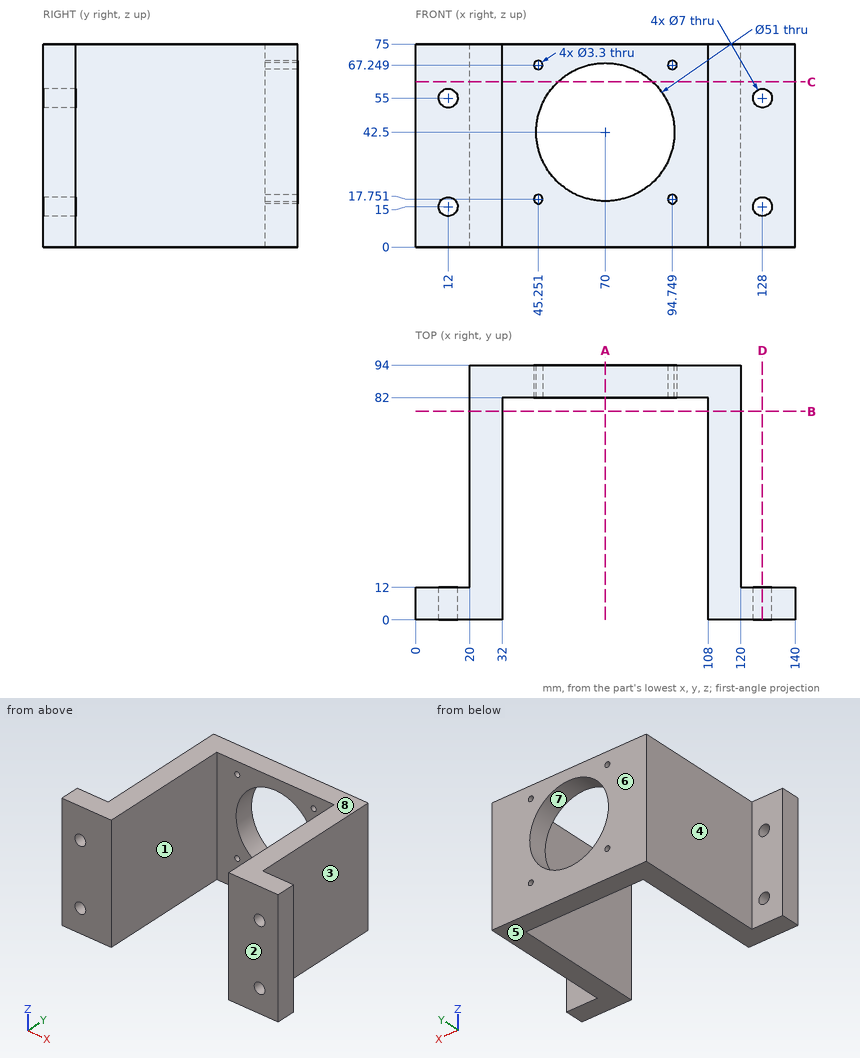
The figure shows three views and two pictorial views of one solid part (mm, origin at its lowest corner). Answer the questions. A direction names the side the tool comes from. Round coordinates to 2 decimals unless told otherwise and drop trailing zeros. Order: outer loops, then holes, each group sorted by start corner. A loop starts at its lowest first (then second) coordinate and runs counter-clockwise, first axis right, second up. Notation, with made-up numbers: M 23.5,43 L 55.5,43 A20 ccw 55.5,61 Z; hole C 25.5,17 d3. An arc over 180 degrees is marked long. Answer in a Markdown table with one row per item. Add a question column.
1) The part is cut by section B-B on y = 77. Determine the outline of the cut face in (x, z), plus the area to 3 significant figures.
2) The part is cut by section D-D on x = 128. Determine the outline of the cut face in (y, z).
3) Which of the six approach directions +Z, -Z, +X, -X, +Y, -Y give full straight-line access (tool end or side, diameter ignored) to the marked faces 1, 2, 3, 4 and 5?
4) The part is cut by section C-C on z = 61. Determine the outline of the cut face in (x, y), plus the area to 3 significant figures.
5) Flat-ended cylindrical pins translate along their axes: pin 1 Ø9 at (x, z) = (128, 55) entering from +Y; pin 2 Ø3 at (y, z) = (25, 25) entering from +X. Find the tip coordinate at first contact, or state that the pin passes through.
6) Determine the mould class of the marked faces 6, 7 and 8 for opening direction Z: pulls with the +Z half, pulls with the -Z half, needs draft (parallel to the pull), parting line crosses it, or undercut.
7) Consider line 1 along X through (y, z) = (5, 15); line 2 along X through (y, z) = (50.5, 69); line 3 along Y through (x, z) = (40, 53.5). Determine where each line is inside the solid, lowest interval first. Write a range as from..to.
8) The part is cut by section A-A on x = 70. Determine the outline of the cut face in (y, z).
Findings below:
| question | item | result |
|---|---|---|
| 1 | outline | M 20,0 L 32,0 L 32,75 L 20,75 Z; M 108,0 L 120,0 L 120,75 L 108,75 Z |
| 1 | area | 1,800 mm² |
| 2 | outline | M 0,0 L 12,0 L 12,11.5 L 0,11.5 Z; M 0,18.5 L 12,18.5 L 12,51.5 L 0,51.5 Z; M 0,58.5 L 12,58.5 L 12,75 L 0,75 Z |
| 3 | face 1 | +Z, -Z, -Y |
| 3 | face 2 | +Z, -Z, +X, -X, -Y |
| 3 | face 3 | +Z, -Z, +X, +Y |
| 3 | face 4 | +Z, -Z, -X, +Y |
| 3 | face 5 | -Z, +X, -X, +Y, -Y |
| 4 | outline | M 0,0 L 32,0 L 32,82 L 52.45,82 L 52.45,94 L 20,94 L 20,12 L 0,12 Z; M 87.55,82 L 108,82 L 108,0 L 140,0 L 140,12 L 120,12 L 120,94 L 87.55,94 Z |
| 4 | area | 3,230 mm² |
| 5 | pin 1 | stops at y = 12 |
| 5 | pin 2 | stops at x = 120 |
| 6 | face 6 | needs draft |
| 6 | face 7 | undercut |
| 6 | face 8 | pulls with the +Z half |
| 7 | line 1 | x = 0..8.5, 15.5..32, 108..124.5, 131.5..140 |
| 7 | line 2 | x = 20..32, 108..120 |
| 7 | line 3 | y = 82..94 |
| 8 | outline | M 82,0 L 94,0 L 94,17 L 82,17 Z; M 82,68 L 94,68 L 94,75 L 82,75 Z |
